Input: dimensioned drawing with shaded views. Units: mm. Origin: part minimum x, y, z. A direction names the side the tool comes from. Round coordinates to 2 decimals unless told otherwise and drop trailing zeros. Order: outer loops, then holes, each group sorted by start corner. A loop starts at its lowest first (then second) coordinate and runs counter-clockwise, first axis right, second up. Notation, with made-up numbers: (26.25, 54.5) -> (31.25, 54.5) arc R14 cw to (31.25, 70.5) -> close; hole circle Ø9 at (53, -18). An arc over 180 degrees is marked (long way). Use a Markdown table: item, result. Add a question column.
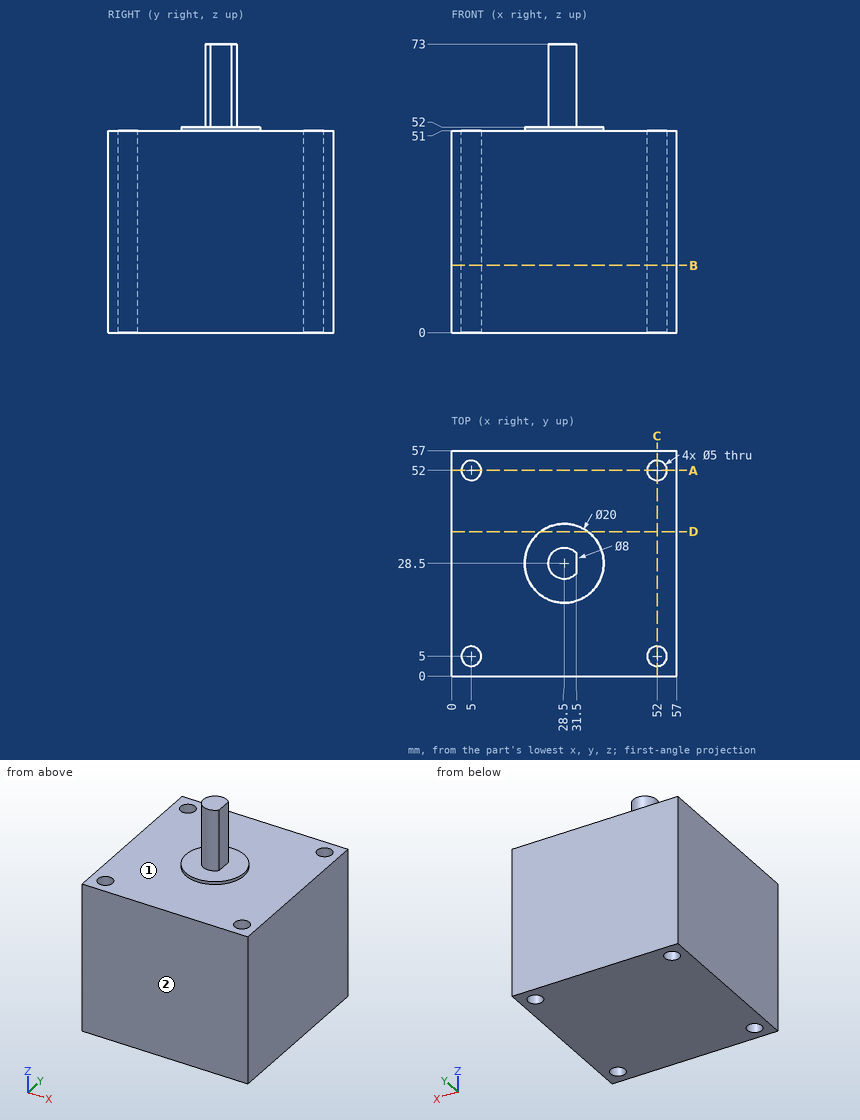
1) Reachability of the marked faces 1 and 2 from +Z, -Z, +X, -X, +Y, -Y: full face, straight path, thin tool, end or side. Return the list, or none.
2) Section A-A on y = 52. Output: boundary loops of the cut face in (x, z).
3) First-contact query: pin 1 Ø6 at (x, y) = (52, 52) entering from +Z; pin 2 Ø4 at (y, z) = (29.5, 58.5) entering from +X. Flat tips, straight axial feed; report the tip coordinate or a pass-through.
4) Section D-D on y = 36.5. Output: boundary loops of the cut face in (x, z).
5) Line query: probe 1 along Y at (x, z) = (52, 38); probe 2 along Y at (x, z) = (53.5, 26); probe 3 along Z at (x, y) = (13, 27.5). Output: solid intervals per line, ascending. Write a range as from..to.
6) Section B-B on z = 17. Output: boundary loops of the cut face in (x, y).
Conclusion:
| question | item | result |
|---|---|---|
| 1 | face 1 | +Z |
| 1 | face 2 | +Z, -Z, +X, -X, -Y |
| 2 | outline | (0, 0) -> (2.5, 0) -> (2.5, 51) -> (0, 51) -> close; (7.5, 0) -> (49.5, 0) -> (49.5, 51) -> (7.5, 51) -> close; (54.5, 0) -> (57, 0) -> (57, 51) -> (54.5, 51) -> close |
| 3 | pin 1 | stops at z = 51 |
| 3 | pin 2 | stops at x = 31.5 |
| 4 | outline | (0, 0) -> (57, 0) -> (57, 51) -> (34.5, 51) -> (34.5, 52) -> (22.5, 52) -> (22.5, 51) -> (0, 51) -> close |
| 5 | probe 1 | y = 0..2.5, 7.5..49.5, 54.5..57 |
| 5 | probe 2 | y = 0..3, 7..50, 54..57 |
| 5 | probe 3 | z = 0..51 |
| 6 | outline | (0, 0) -> (57, 0) -> (57, 57) -> (0, 57) -> close; hole circle Ø5 at (5, 5); hole circle Ø5 at (5, 52); hole circle Ø5 at (52, 5); hole circle Ø5 at (52, 52) |
